CAD build for the part. Positions are in the model's coordinates, mm. Face numbers are marked on the shaded views. Coordinates: 2 decimals unless noted, no trailing zeros. Order: outer loops, then holes, each group sorted by start corner. A loop starts at its lowest first (then second) coordinate and runs counter-clockwise, first axis right, second up. Notation, with made-up numbers: (-17.5, 37.5) - (15.5, 37.5) arc R25 ccw to (15.5, 51.5) - close; hole circle Ø11 at (21, -11). An arc over 180 degrees is marked (long way). Return JSON: item names as keys, results as strings.
from build123d import *
from build123d.topology import SkipClean

# Parameters (mm, degrees)
BASE_FLANGE_SKETCH_R     = 6
BASE_FLANGE_DEPTH        = 8
TUBE_START               = 88
TUBE_SKETCH_R            = 37.5
TUBE_75_DEPTH            = 88
BORE_SKETCH_R            = 28
BORE_56_DEPTH            = 76
SPIGOT_SKETCH_R          = 19
SPIGOT_38_DEPTH          = 6
SPIGOT_HOLE_SKETCH_R     = 11
SPIGOT_HOLE_22_DEPTH     = 22
BORE_STEP_SKETCH_R       = 22.5
BORE_STEP_45_DEPTH       = 12
CROSS_HOLE_12_DEPTH      = 134.912284724
CROSS_HOLE_12_DEPTH_BACK = 134.912284724
CROSS_HOLE_SKETCH_R      = 6


with BuildPart() as part:
    # Base Flange Sketch → Base Flange (new, symmetric)
    with BuildSketch(Plane(origin=(0, 0, 0), x_dir=(1, 0, 0), z_dir=(0, 1, 0))):
        with BuildLine():
            Line((-62.126086957, -27.615200877), (-6.195652174, -36.984644032))
            ThreePointArc((-6.195652174, -36.984644032), (0, -37.5), (6.195652174, -36.984644032))
            Line((6.195652174, -36.984644032), (62.126086957, -27.615200877))
            ThreePointArc((62.126086957, -27.615200877), (85.5, 0), (62.126086957, 27.615200877))
            Line((62.126086957, 27.615200877), (6.195652174, 36.984644032))
            ThreePointArc((6.195652174, 36.984644032), (0, 37.5), (-6.195652174, 36.984644032))
            Line((-6.195652174, 36.984644032), (-62.126086957, 27.615200877))
            ThreePointArc((-62.126086957, 27.615200877), (-85.5, 0), (-62.126086957, -27.615200877))
        make_face()
        with Locations(Location((-57.5, 0, 0), (0, 0, 270))):
            Circle(BASE_FLANGE_SKETCH_R, mode=Mode.SUBTRACT)
        with Locations(Location((57.5, 0, 0), (0, 0, 270))):
            Circle(BASE_FLANGE_SKETCH_R, mode=Mode.SUBTRACT)
    extrude(amount=BASE_FLANGE_DEPTH, both=True)

    # Tube Sketch → Tube Ø75 (add)
    with SkipClean():  # the faces are left unmerged after this step: merging them gives an invalid solid
        with BuildSketch(Plane(origin=(0, 8, 0), x_dir=(1, 0, 0), z_dir=(0, 1, 0)).offset(TUBE_START)):
            with Locations(Location((0, 0, 0), (0, 0, 99.5098634))):
                Circle(TUBE_SKETCH_R)
        extrude(amount=-TUBE_75_DEPTH)

    # Bore Sketch → Bore Ø56 (cut)
    with SkipClean():  # the faces are left unmerged after this step: merging them gives an invalid solid
        with BuildSketch(Plane(origin=(0, 96, 0), x_dir=(1, 0, 0), z_dir=(0, 1, 0))):
            with Locations(Location((0, 0, 0), (0, 0, 270))):
                Circle(BORE_SKETCH_R)
        extrude(amount=-BORE_56_DEPTH, mode=Mode.SUBTRACT)

    # Spigot Sketch → Spigot Ø38 (add)
    with SkipClean():  # the faces are left unmerged after this step: merging them gives an invalid solid
        with BuildSketch(Plane.XZ.offset(8)):
            with Locations(Location((0, 0, 0), (0, 0, 270))):
                Circle(SPIGOT_SKETCH_R)
        extrude(amount=SPIGOT_38_DEPTH)

    # Spigot Hole Sketch → Spigot Hole Ø22 (cut)
    with SkipClean():  # the faces are left unmerged after this step: merging them gives an invalid solid
        with BuildSketch(Plane.XZ.offset(14)):
            with Locations(Location((0, 0, 0), (0, 0, 270))):
                Circle(SPIGOT_HOLE_SKETCH_R)
        extrude(amount=-SPIGOT_HOLE_22_DEPTH, mode=Mode.SUBTRACT)

    # Bore Step Sketch → Bore Step Ø45 (cut)
    with SkipClean():  # the faces are left unmerged after this step: merging them gives an invalid solid
        with BuildSketch(Plane(origin=(0, 20, 0), x_dir=(1, 0, 0), z_dir=(0, 1, 0))):
            with Locations(Location((0, 0, 0), (0, 0, 270))):
                Circle(BORE_STEP_SKETCH_R)
        extrude(amount=-BORE_STEP_45_DEPTH, mode=Mode.SUBTRACT)

    # Cross Hole Sketch → Cross Hole Ø12 (cut, two sides: drawn at the far end of the back side and taken through both)
    with SkipClean():  # the faces are left unmerged after this step: merging them gives an invalid solid
        with BuildSketch(Plane(origin=(0, 0, 0), x_dir=(0, 0, -1), z_dir=(1, 0, 0)).offset(-CROSS_HOLE_12_DEPTH_BACK)):
            with Locations((0, 43)):
                Circle(CROSS_HOLE_SKETCH_R)
        extrude(amount=CROSS_HOLE_12_DEPTH + CROSS_HOLE_12_DEPTH_BACK, mode=Mode.SUBTRACT)


solid = part.part
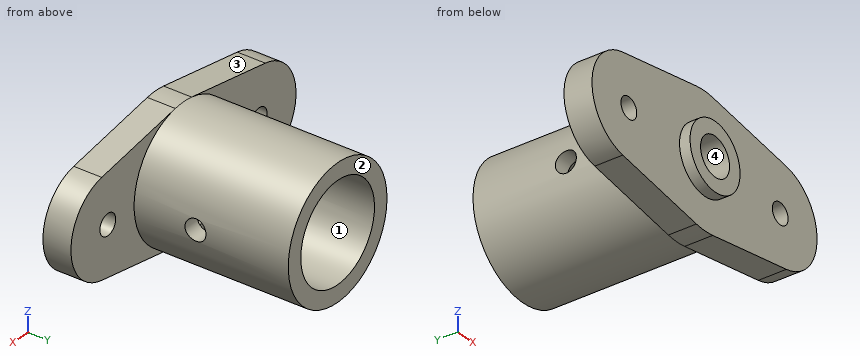
Item 1: Band-saw the part on D-D, the plane x = 60. List the corners of the cut face in (y, z).
Findings below:
{"outline": "(-8, -27.97) - (8, -27.97) - (8, -5.45) - (-8, -5.45) - close; (-8, 5.45) - (8, 5.45) - (8, 27.97) - (-8, 27.97) - close"}
Item 2: Drop flat-ended pins along their axis: P1, Ø5, axis at x = -14, z = 23.5, coming from the +Y side; P2, Ø2, axis at y = 22, z = -4, coming from the -X side; P3, Ø2, axis at x = 19, z = 11, coming from the -Y side; P4, Ø14, axis at y = 43, z = 0, coming from the -X side. Give the stop position or say it passes through.
Findings below:
{"P1": "stops at y = 96", "P2": "stops at x = -37.38", "P3": "stops at y = -8", "P4": "stops at x = -37.5"}
Item 3: Band-saw the part on A-A, the plane x = 0. List the corners of the cut face in (y, z).
Findings below:
{"outline": "(-14, -19) - (-8, -19) - (-8, -37.5) - (96, -37.5) - (96, -28) - (20, -28) - (20, -22.5) - (8, -22.5) - (8, -11) - (-14, -11) - close; (-14, 11) - (8, 11) - (8, 22.5) - (20, 22.5) - (20, 28) - (96, 28) - (96, 37.5) - (-8, 37.5) - (-8, 19) - (-14, 19) - close"}
Item 4: Band-saw the part on C-C, the plane y = 33. List the corners of the cut face in (x, z), then the cut area to 3 significant figures.
Findings below:
{"outline": "circle Ø75 at (0, 0); hole circle Ø56 at (0, 0)", "area": "1,950 mm²"}
Item 5: Wall check: L1, parallel to Y at x = -32, z = 0; L2, parallel to Y at x = 5, z = 14; L3, parallel to Y at x = -41, z = -6. Give the ranges that are in metal, low to high. Write a range as [from, to].
Findings below:
{"L1": "y = [-8, 37], [49, 96]", "L2": "y = [-14, 8]", "L3": "y = [-8, 8]"}
Item 6: Mould opens along X. For the marked faces 1, 2, 3 and 4 say: released by +X, released by -X, zero draft, split by the parting line, or undercut.
Findings below:
{"face 1": "undercut", "face 2": "zero draft", "face 3": "released by -X", "face 4": "undercut"}
Item 7: Band-saw the part on B-B, the plane z = -8.5. List the corners of the cut face in (x, y).
Findings below:
{"outline": "(-84.18, -8) - (-16.99, -8) - (-16.99, -14) - (-6.98, -14) - (-6.98, 8) - (-20.83, 8) - (-20.83, 20) - (-26.68, 20) - (-26.68, 96) - (-36.52, 96) - (-36.52, 8) - (-84.18, 8) - close; (6.98, -14) - (16.99, -14) - (16.99, -8) - (84.18, -8) - (84.18, 8) - (36.52, 8) - (36.52, 96) - (26.68, 96) - (26.68, 20) - (20.83, 20) - (20.83, 8) - (6.98, 8) - close"}
